from build123d import *

# Parameters (mm, degrees)
CUT_EXTRUDE1_DEPTH      = 8
CUT_EXTRUDE1_DEPTH_BACK = 8


with BuildPart() as part:
    # Sketch1 → Revolve1 (revolve)
    with BuildSketch(Plane.XY, mode=Mode.PRIVATE) as revolve1_sk:
        Polygon((5.435884786, 0), (4.5, 1.621), (-3.121, 1.621), (-3.5, 2), (-3.5, 4), (25, 4), (25, 8), (30, 8), (30, 0), align=None)
    revolve(revolve1_sk.sketch.rotate(Axis((30, 0, 0), (-1, 0, 0)), 180), axis=Axis((30, 0, 0), (-1, 0, 0)))

    # Sketch2 → Cut-Extrude1 (cut, two sides: drawn at the far end of the back side and taken through both)
    with BuildSketch(Plane(origin=(0, 0, 0), x_dir=(1, 0, 0), z_dir=(0, 1, 0)).offset(-CUT_EXTRUDE1_DEPTH_BACK)):
        Polygon((-8.5, 8), (-8.5, -8), (5, -8), (0, -3), (-3.5, -3), (-3.5, 3), (0, 3), (5, 8), align=None)
    extrude(amount=CUT_EXTRUDE1_DEPTH + CUT_EXTRUDE1_DEPTH_BACK, mode=Mode.SUBTRACT)


solid = part.part
Geometry check sheet. Reference: the model listing, model coordinates, mm. A direction names the side the tool comes from. Round coordinates to 2 decimals unless told otherwise and drop trailing zeros. Order: outer loops, then holes, each group sorted by start corner. A loop starts at its lowest first (then second) coordinate and runs counter-clockwise, first axis right, second up. Notation, with made-up numbers: (63, -18) -> (81, -18) arc R14 cw to (81, -8) -> close; hole circle Ø2 at (84.5, 52.5). An arc over 180 degrees is marked (long way). Use one line per item in the form item = value.
1. Cross-section at A-A, the plane y = -3. Enter the section's corners in (x, z), plus the area to 3 significant figures.
Working result:
outline = (-3.5, -2.65) -> (25, -2.65) -> (25, -7.42) -> (30, -7.42) -> (30, 7.42) -> (25, 7.42) -> (25, 2.65) -> (-3.5, 2.65) -> close
area = 225 mm^2
2. Scan lines: line 1 along Z through (x, y) = (1, 0); line 2 along Z through (x, y) = (24.5, -0.25); line 3 along Z through (x, y) = (0.25, 0). Record each from-to range of solid material in increasing order. Write a range as from..to.
Working result:
line_1 = -4..-1.62, 1.62..4
line_2 = -3.99..3.99
line_3 = -3.25..-1.62, 1.62..3.25
3. Mould release check, pull along Y, two halves, no side actions. Record for faces 1 (the face through (5.273, 0.061, -0.275)), 2 (the face through (-3.5, 1, 2)), 3 (the face through (27.54, 1.73, -7.81)): pulls with the +Y half, pulls with the -Y half, needs draft (parallel to the pull), parting line crosses it, or undercut.
Working result:
face_1 = undercut
face_2 = needs draft
face_3 = parting line crosses it
4. Cross-section at D-D, the plane x = 17. Enter the section's corners in (y, z).
Working result:
outline = circle Ø8 at (0, 0)
5. Cross-section at B-B, the plane x = 2. Enter the section's corners in (y, z).
Working result:
outline = circle Ø8 at (0, 0); hole circle Ø3.24 at (0, 0)
6. Set-up check for faces 4 (the face through (30, 0, 0)), 5 (the face through (25, 2, 4)), 6 (the face through (-2, 0, -3)), 7 (the face through (-2, 0, 3)): record each of +Z, -Z, +X, -X, +Y, -Y from which the full face is reachable in a straight line by a thin tool's end or side.
Working result:
face_4 = +Z, -Z, +X, +Y, -Y
face_5 = -X
face_6 = -Z, -X, +Y, -Y
face_7 = +Z, -X, +Y, -Y
7. Cross-section at C-C, the plane z = -2.5. Enter the section's corners in (x, y), plus the area to 3 significant figures.
Working result:
outline = (-3.5, -3.12) -> (25, -3.12) -> (25, -7.6) -> (30, -7.6) -> (30, 7.6) -> (25, 7.6) -> (25, 3.12) -> (-3.5, 3.12) -> close
area = 254 mm^2
8. Go/stop test with flat-tipped pins: pin 1 (8 mm diameter, centred on x = 16, z = -1, fed in from -Y); pin 2 (8 mm diameter, centred on x = 14.5, y = 2, fed in from +Z); pin 3 (1 mm diameter, centred on x = 25.5, y = -4.5, fed in from -Z). Record where each tip stops, or that it passes through.
Working result:
pin_1 = -4
pin_2 = 4
pin_3 = -6.93
